Here's how the part is built. I have some questions about the finished solid (model axes, mm). Face numbers are marked on the shaded views. Round coordinates to 2 decimals unless told otherwise and drop trailing zeros. Order: outer loops, then holes, each group sorted by start corner. A loop starts at its lowest first (then second) coordinate and runs counter-clockwise, first axis right, second up. Notation, with made-up numbers: M 76.25,40 L 118.25,40 A35 cw 118.25,77 Z; hole C 52.5,34.5 d5. An arc over 180 degrees is marked long. Write item = value, one per line. Start each with the question number.
Item 1: Please list where these lines run through material, in increasing order: L1, parallel to X at y = -56, z = 10; L2, parallel to Y at x = 65.5, z = 7.25; L3, parallel to Y at x = 29, z = 4.25.
Item 2: I want a section at A-A, the plane z = 6.5. List the corners of the cut face in (x, y) for me.
Item 3: I'm going to push flat-ended pins straight in: P1, Ø1.5, axis at x = 76.5, z = 10, coming from the +Y side; P2, Ø5, axis at x = 66.5, z = 12.5, coming from the -Y side; P3, Ø7.5, axis at y = -5, z = 10, coming from the +X side; P4, Ø24, axis at x = 45.08, y = -130, coming from the -Z side. Where does each tip first touch, or does it pass through?
Item 4: I want a section at B-B, the plane y = -130. List the corners of the cut face in (x, z) for me.
Item 5: I want a section at D-D, the plane x = 31. List the corners of the cut face in (y, z) for me.
Item 6: I want a section at C-C, the plane x = 56.5. List the corners of the cut face in (y, z) for me.
Item 7: We'd pull the mould along X, two halves only. Please class the marked faces 1, 2, 3 and 4: pulls with the +X half, pulls with the -X half, needs draft (parallel to the pull), parting line crosses it, or undercut.
```python
from build123d import *
from build123d.topology import SkipClean

# Parameters (mm, degrees)
SKETCH_1_R      = 20
EXTRUDE_1_DEPTH = 12
EXTRUDE_2_DEPTH = 10
EXTRUDE_3_DEPTH = 2
SKETCH_5_R      = 20
EXTRUDE_4_DEPTH = 3


with BuildPart() as part:
    # 草图1 → 凸台-拉伸1 (new body)
    with BuildSketch(Plane.XY):
        with BuildLine():
            Line((0, 0), (70, 0))
            Line((70, 0), (70, -15))
            Line((70, -15), (50, -45))
            Line((50, -45), (50, -65.266069056))
            Line((50, -65.266069056), (78.36394873, -107.811992151))
            ThreePointArc((78.36394873, -107.811992151), (80.348920907, -148.874317021), (45.081936956, -170))
            Line((45.081936956, -170), (0, -170))
            Line((0, -170), (0, 0))
        make_face()
        with Locations((45.081936956, -130)):
            Circle(SKETCH_1_R, mode=Mode.SUBTRACT)
    extrude(amount=EXTRUDE_1_DEPTH)

    # 草图3 → 凸台-拉伸2 (add)
    with BuildSketch(Plane.XY.offset(12)):
        with BuildLine():
            Line((50, -45), (50, -55.133034528))
            Line((50, -55.133034528), (52.687024396, -55.133034528))
            ThreePointArc((52.687024396, -55.133034528), (54.694220679, -41.57719354), (60.543560077, -29.184659884))
            Line((60.543560077, -29.184659884), (50, -45))
        make_face()
        with BuildLine():
            Line((52.687024396, -55.133034528), (50, -55.133034528))
            Line((50, -55.133034528), (50, -65.266069056))
            Line((50, -65.266069056), (60.543560077, -81.081409172))
            ThreePointArc((60.543560077, -81.081409172), (54.694220679, -68.688875516), (52.687024396, -55.133034528))
        make_face()
    extrude(amount=-EXTRUDE_2_DEPTH)

    # 草图4 → 凸台-拉伸3 (add)
    with BuildSketch(Plane(origin=(0, 0, 2), x_dir=(-1, 0, 0), z_dir=(0, 0, -1))):
        with BuildLine():
            Line((-60.543560077, -81.081409172), (-50, -65.266069056))
            Line((-50, -65.266069056), (-50, -45))
            Line((-50, -45), (-60.543560077, -29.184659884))
            ThreePointArc((-60.543560077, -29.184659884), (-52.687024396, -55.133034528), (-60.543560077, -81.081409172))
        make_face()
    extrude(amount=EXTRUDE_3_DEPTH)

    # 草图5 → 凸台-拉伸4 (add)
    with SkipClean():  # the faces are left unmerged after this step: merging them gives an invalid solid
        with BuildSketch(Plane.XY.offset(12)):
            with BuildLine():
                Line((0, 0), (0, -170))
                Line((0, -170), (45.081936956, -170))
                ThreePointArc((45.081936956, -170), (80.348920907, -148.874317021), (78.36394873, -107.811992151))
                Line((78.36394873, -107.811992151), (60.543560077, -81.081409172))
                ThreePointArc((60.543560077, -81.081409172), (52.687024396, -55.133034528), (60.543560077, -29.184659884))
                Line((60.543560077, -29.184659884), (70, -15))
                Line((70, -15), (70, 0))
                Line((70, 0), (0, 0))
            make_face()
            with Locations((45.081936956, -130)):
                Circle(SKETCH_5_R, mode=Mode.SUBTRACT)
        extrude(amount=EXTRUDE_4_DEPTH)


solid = part.part
```
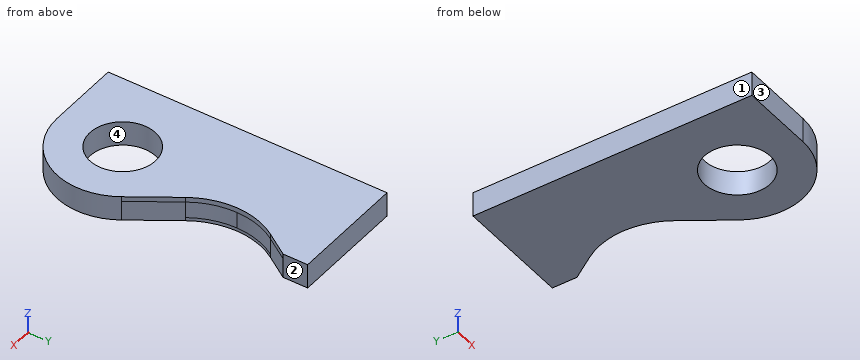
Filled in:
q1.L1 = 0 to 52.7
q1.L2 = -164.4 to -88.52, -21.75 to 0
q1.L3 = -170 to -141.89, -118.11 to 0
q2.outline = M 0,-170 L 45.08,-170 A40 ccw 78.36,-107.81 L 60.54,-81.08 A46.78 cw 60.54,-29.18 L 70,-15 L 70,0 L 0,0 Z; hole C 45.08,-130 d40
q3.P1 = -103.89
q3.P2 = -165.24
q3.P3 = 70
q3.P4 = through
q4.outline = M 0,0 L 25.08,0 L 25.08,15 L 0,15 Z; M 65.08,0 L 85.08,0 L 85.08,15 L 65.08,15 Z
q5.outline = M -170,0 L -144.2,0 L -144.2,15 L -170,15 Z; M -115.8,0 L 0,0 L 0,15 L -115.8,15 Z
q6.outline = M -168.34,0 L -146.42,0 L -146.42,15 L -168.34,15 Z; M -113.58,0 L -73.63,0 L -73.63,15 L -113.58,15 Z; M -36.63,0 L 0,0 L 0,15 L -36.63,15 Z
q7.face_1 = pulls with the -X half
q7.face_2 = pulls with the +X half
q7.face_3 = needs draft
q7.face_4 = undercut
